```python
from build123d import *

# Parameters (mm, degrees)
EXTRUDE_1_DEPTH     = 148
SKETCH_2_R          = 2.25
CUT_EXTRUDE_1_DEPTH = 10


with BuildPart() as part:
    # 草图1 → 凸台-拉伸1 (new, symmetric)
    with BuildSketch(Plane.XY):
        Polygon((-37.5, 0), (-39.5, 0), (-39.5, 4.3), (-30, 6), (30, 6), (39.5, 4.3), (39.5, 0), (37.5, 0), (37.5, 2.122105263), (29.8, 3.5), (-29.8, 3.5), (-37.5, 2.122105263), align=None)
    extrude(amount=EXTRUDE_1_DEPTH, both=True)

    # 草图2 → 切除-拉伸1 (cut)
    with BuildSketch(Plane(origin=(0, 6, 0), x_dir=(1, 0, 0), z_dir=(0, 1, 0))):
        with Locations(Location((-20, -143, 0), (0, 0, 270))):
            Circle(SKETCH_2_R)
        with Locations(Location((20, -143, 0), (0, 0, 270))):
            Circle(SKETCH_2_R)
    cut_extrude_1 = extrude(amount=-CUT_EXTRUDE_1_DEPTH, mode=Mode.SUBTRACT)

    # 镜向1: 切除-拉伸1 across plane
    add(cut_extrude_1.mirror(Plane.XY), mode=Mode.SUBTRACT)


solid = part.part
```
Geometry: final body of the model. Coordinates: model frame, mm. A direction names the side the tool comes from. Round coordinates to 2 decimals unless told otherwise and drop trailing zeros. Write each loop counter-clockwise with the first axis right and the second up, starting at its lowest first coordinate (ties: lowest second). Pieces come first, ordered by that corner, then holes.
Item 1: Mould query, pull axis X, two halves, no side actions, for faces 1 (the face through (-33.6, 2.82, 2.07)), 2 (the face through (1, 4, 148)), 3 (the face through (34.684, 5.162, 2.072)). Classes: +X half, -X half, draft (parallel to the pull), parting line (faces both ways), or undercut.
Item 2: Section query B-B (x = -9.5). Return loops of the section in (y, z), plus the area to 3 significant figures.
Item 3: Section query A-A (z = 68). Return loops of the section in (x, y), plus the area to 3 significant figures.
Item 4: Set-up query: faces 4 (the face through (0, 6, 2)), 5 (the face through (33.704, 2.801, 2.072)). Return all of +Z, -Z, +X, -X, +Y, -Y with unobstructed straight access to the full face (end or side cutting, diameter ignored); none if empty.
Item 5: Material intervals for L1, parallel to X at y = 4.1, z = 143; L2, parallel to X at y = 1.9, z = 117.5; L3, parallel to Y at x = 29, z = 32.5, sorted ascending.
Item 6: Pin query (flat end, axial travel): P1, Ø1, axis at x = 19, y = 2.5, coming from the -Z side; P2, Ø6, axis at x = 20, z = 143, coming from the -Y side. Return the tip coordinate at first contact, or that it passes through.
Completed:
1. face 1: undercut
1. face 2: draft
1. face 3: +X half
2. outline: (3.5, -148) - (6, -148) - (6, 148) - (3.5, 148) - close
2. area: 740 mm2
3. outline: (-39.5, 0) - (-37.5, 0) - (-37.5, 2.12) - (-29.8, 3.5) - (29.8, 3.5) - (37.5, 2.12) - (37.5, 0) - (39.5, 0) - (39.5, 4.3) - (30, 6) - (-30, 6) - (-39.5, 4.3) - close
3. area: 206 mm2
4. face 4: +Z, -Z, +X, -X, +Y
4. face 5: +Z, -Z, -Y
5. L1: x = -39.5 to -22.25, -17.75 to 17.75, 22.25 to 39.5
5. L2: x = -39.5 to -37.5, 37.5 to 39.5
5. L3: y = 3.5 to 6
6. P1: passes through
6. P2: stops at y = 3.5
